CAD build for the part. Positions are in the model's coordinates, mm. A direction names the side the tool comes from. Coordinates: 2 decimals unless noted, no trailing zeros. Loops run counter-clockwise (first coordinate to the right, second up) from the corner with the lowest first, then second, coordinate; pieces in that order, holes last. Notation, with made-up numbers: M 26.5,53 L 30.5,53 A18 ccw 30.5,79 Z; hole C 60,26 d8. An arc over 180 degrees is marked long. Answer as a JSON object with one key per item and string values. Group by question number.
```python
from build123d import *

# Parameters (mm, degrees)
SKETCH1_W           = 100
SKETCH1_H           = 70
BOSS_EXTRUDE1_DEPTH = 10
SKETCH2_R           = 5
CUT_EXTRUDE1_DEPTH  = 10
SKETCH3_W           = 150
SKETCH3_H           = 70
BOSS_EXTRUDE2_DEPTH = 10
CUT_EXTRUDE2_DEPTH  = 50


with BuildPart() as part:
    # Sketch1 → Boss-Extrude1 (new body)
    with BuildSketch(Plane.XY):
        Rectangle(SKETCH1_W, SKETCH1_H)
    extrude(amount=BOSS_EXTRUDE1_DEPTH)

    # Sketch2 → Cut-Extrude1 (cut)
    with BuildSketch(Plane.XY.offset(10)):
        with Locations((-30, 0)):
            Circle(SKETCH2_R)
        with Locations((30, 0)):
            Circle(SKETCH2_R)
    extrude(amount=-CUT_EXTRUDE1_DEPTH, mode=Mode.SUBTRACT)

    # Sketch3 → Boss-Extrude2 (add)
    with BuildSketch(Plane(origin=(50, 0, 0), x_dir=(0, 0, -1), z_dir=(1, 0, 0))):
        with Locations((-75, 0)):
            Rectangle(SKETCH3_W, SKETCH3_H)
    extrude(amount=BOSS_EXTRUDE2_DEPTH)

    # Sketch7 → Cut-Extrude2 (cut)
    with BuildSketch(Plane.ZY.offset(-50)):
        with BuildLine():
            Line((138.396107193, -4.795166993), (37.396107193, -4.795166993))
            ThreePointArc((37.396107193, -4.795166993), (34.214126678, -3.477147509), (32.896107193, -0.295166993))
            Line((32.896107193, -0.295166993), (32.896107193, 0.704833007))
            ThreePointArc((32.896107193, 0.704833007), (34.214126678, 3.886813522), (37.396107193, 5.204833007))
            Line((37.396107193, 5.204833007), (138.396107193, 5.204833007))
            ThreePointArc((138.396107193, 5.204833007), (141.578087709, 3.886813522), (142.896107193, 0.704833007))
            Line((142.896107193, 0.704833007), (142.896107193, -0.295166993))
            ThreePointArc((142.896107193, -0.295166993), (141.578087709, -3.477147509), (138.396107193, -4.795166993))
        make_face()
    extrude(amount=-CUT_EXTRUDE2_DEPTH, mode=Mode.SUBTRACT)


solid = part.part
```
Item 1: Slice it at A-A, the plane x = 30. Write the cut outline in (y, z), then the cut area to 3 significant figures.
Item 2: Pin check, flat tips, straight feed: pin 1 (1.5 mm diameter, centred on y = -16.5, z = 29.5, fed in from -X); pin 2 (2 mm diameter, centred on x = 35.5, y = -25, fed in from +Z). Stop position of each tip, or through.
Item 3: Drill centre lines: L1, parallel to Y at x = -30, z = 6.25; L2, parallel to Z at x = 19, y = 27.5; L3, parallel to X at y = 21, z = 83. Where is each one in solid material? Low to high. Write a range as from..to.
Item 4: Tool access for faces 5 (the flat face through (55, 0, 150)), 6 (the flat face through (55, -4.795, 89)), 7 (the flat face through (50, 8, 81)): list every direction of +Z, -Z, +X, -X, +Y, -Y with a clear straight run to the whole face (end or side of a thin tool).
Item 5: Pull direction Z, two halves, no side cores. Call faces 1 (the cylindrical face through (54.93, -3.442, 141.613)), 2 (the flat face through (-1, 0, 10)), 3 (the flat face through (54, -35, 42)), 4 (the cylindrical face through (54.93, 3.922, 141.543)): released by +Z, released by -Z, zero draft, split by the parting line, or undercut.
Item 6: Slice it at D-D, the plane y = 29. Write the cut outline in (x, z), then the cut area to 3 significant figures.
Item 7: Slice it at B-B, the plane z = 100.5. Write the cut outline in (x, y), then the cut area to 3 significant figures.
Item 8: Slice it at C-C, the plane y = -2. Write the cut outline in (x, z), then the cut area to 3 significant figures.
Computed:
{
 "1": {"outline": "M -35,0 L -5,0 L -5,10 L -35,10 Z; M 5,0 L 35,0 L 35,10 L 5,10 Z", "area": "600 mm2"},
 "2": {"pin 1": "x = 50", "pin 2": "z = 10"},
 "3": {"L1": "-35..-5, 5..35", "L2": "0..10", "L3": "50..60"},
 "4": {"face 5": "+Z, +X, -X, +Y, -Y", "face 6": "+X, -X", "face 7": "+Z, -X, +Y, -Y"},
 "5": {"face 1": "undercut", "face 2": "released by +Z", "face 3": "zero draft", "face 4": "undercut"},
 "6": {"outline": "M -50,0 L 60,0 L 60,150 L 50,150 L 50,10 L -50,10 Z", "area": "2,500 mm2"},
 "7": {"outline": "M 50,-35 L 60,-35 L 60,-4.8 L 50,-4.8 Z; M 50,5.2 L 60,5.2 L 60,35 L 50,35 Z", "area": "600 mm2"},
 "8": {"outline": "M -50,0 L -34.58,0 L -34.58,10 L -50,10 Z; M -25.42,0 L 25.42,0 L 25.42,10 L -25.42,10 Z; M 34.58,0 L 60,0 L 60,33.23 L 50,33.23 L 50,10 L 34.58,10 Z; M 50,142.56 L 60,142.56 L 60,150 L 50,150 Z", "area": "1,220 mm2"}
}
